```python
from build123d import *

# Parameters (mm, degrees)
SKETCH_1_W          = 200
SKETCH_1_H          = 200
EXTRUDE_1_DEPTH     = 25
SKETCH_2_W          = 150
SKETCH_2_H          = 150
EXTRUDE_2_DEPTH     = 154
SKETCH_3_R          = 60
EXTRUDE_3_DEPTH     = 154
FILLET_1_R          = 10
SKETCH_4_R          = 50
EXTRUDE_4_DEPTH     = 100
SKETCH_5_R          = 50
SKETCH_5_R_2        = 45
EXTRUDE_5_DEPTH     = 100
SKETCH_6_R          = 48
CUT_EXTRUDE_1_DEPTH = 100


with BuildPart() as part:
    # 草图1 → 凸台-拉伸1 (new body)
    with BuildSketch(Plane.XY):
        Rectangle(SKETCH_1_W, SKETCH_1_H)
    extrude(amount=EXTRUDE_1_DEPTH)

    # 草图2 → 凸台-拉伸2 (add)
    with BuildSketch(Plane.XY.offset(25)):
        Rectangle(SKETCH_2_W, SKETCH_2_H)
    extrude(amount=EXTRUDE_2_DEPTH)

    # 草图3 → 凸台-拉伸3 (add)
    with BuildSketch(Plane(origin=(-75, 0, 0), x_dir=(0, 0, -1), z_dir=(1, 0, 0))):
        with Locations((-105, -5)):
            Circle(SKETCH_3_R)
    extrude(amount=-EXTRUDE_3_DEPTH)

    # 圆角1
    fillet_1_edges = [part.edges().sort_by_distance(p)[0] for p in [
        (-229, -5, 165),
    ]]
    fillet(fillet_1_edges, radius=FILLET_1_R)

    # 草图4 → 凸台-拉伸4 (add)
    with BuildSketch(Plane.XY.offset(179)):
        Circle(SKETCH_4_R)
    extrude(amount=EXTRUDE_4_DEPTH)

    # 草图5 → 凸台-拉伸5 (add)
    with BuildSketch(Plane(origin=(0, 75, 0), x_dir=(1, 0, 0), z_dir=(0, 1, 0))):
        with Locations(Location((0, -85, 0), (0, 0, 90))):
            Circle(SKETCH_5_R)
        with Locations(Location((0, -85, 0), (0, 0, 270))):
            Circle(SKETCH_5_R_2, mode=Mode.SUBTRACT)
    extrude(amount=EXTRUDE_5_DEPTH)

    # 草图6 → 切除-拉伸1 (cut)
    with BuildSketch(Plane.XY.offset(279)):
        Circle(SKETCH_6_R)
    extrude(amount=-CUT_EXTRUDE_1_DEPTH, mode=Mode.SUBTRACT)


solid = part.part
```
Could you check a few things on this model? Use its own coordinates, in mm. A direction names the side the tool comes from. Round coordinates to 2 decimals unless told otherwise and drop trailing zeros. Order: outer loops, then holes, each group sorted by start corner. A loop starts at its lowest first (then second) coordinate and runs counter-clockwise, first axis right, second up. Notation, with made-up numbers: (19.5, -26.5) -> (38.5, -26.5) arc R7 ccw to (38.5, -20.5) -> close; hole circle Ø1 at (8, 20). An arc over 180 degrees is marked (long way). One line per question, with ' | ' between items.
Q1. We'd pull the mould along X, two halves only. Please class faces 1 (the face through (-47.954, 2.11, 229.7)), 2 (the face through (1.979, 124.3, 40.044)), 3 (the face through (-1, 1, 0)), 4 (the face through (47.69, 15.02, 228.3)): released by +X, released by -X, zero draft, split by the parting line, or undercut.
Computed values:
face 1: undercut | face 2: undercut | face 3: zero draft | face 4: split by the parting line
Q2. If we section it at C-C on z = 219: Write out the boundary of the cut face in (x, y), plus the area to 3 significant figures.
Computed values:
outline: circle Ø100 at (0, 0); hole circle Ø96 at (0, 0) | area: 616 mm²
Q3. Which directions (+Z, -Z, +X, -X, +Y, -Y) give clear straight access to the entire face, cutting with the end or side of a thin tool? Please do faces 5 (the face through (-90, 1, 25)), 6 (the face through (-1, 51, 179)), 7 (the face through (-145.99, -2.36, 164.94)).
Computed values:
face 5: none | face 6: +Z | face 7: -X
Q4. If we section it at D-D on y = 113.5: Write out the boundary of the cut face in (x, z).
Computed values:
outline: circle Ø100 at (0, 85); hole circle Ø90 at (0, 85)
Q5. If we section it at A-A on y = 84: Write out the boundary of the cut face in (x, z), plus the area to 3 significant figures.
Computed values:
outline: (-100, 0) -> (100, 0) -> (100, 25) -> (-100, 25) -> close; circle Ø100 at (0, 85); hole circle Ø90 at (0, 85) | area: 6,490 mm²
Q6. I'm going to push flat-ended pins straight in: pin 1 (7.5 mm diameter, centred on x = -22, z = 11, fed in from +Y); pin 2 (3 mm diameter, centred on y = 117, z = 72.5, fed in from -X) (3 decimals); pin 3 (12.5 mm diameter, centred on y = 20.5, z = 9.5, fed in from -X). Where does each tip first touch, or does it pass through?
Computed values:
pin 1: y = 100 | pin 2: x = -48.775 | pin 3: x = -100
Q7. If we section it at B-B on x = 0: Write out the boundary of the cut face in (y, z).
Computed values:
outline: (-100, 0) -> (100, 0) -> (100, 25) -> (75, 25) -> (75, 35) -> (175, 35) -> (175, 40) -> (75, 40) -> (75, 130) -> (175, 130) -> (175, 135) -> (75, 135) -> (75, 179) -> (50, 179) -> (50, 279) -> (48, 279) -> (48, 179) -> (-48, 179) -> (-48, 279) -> (-50, 279) -> (-50, 179) -> (-75, 179) -> (-75, 25) -> (-100, 25) -> close
Q8. If I drill on line 1 (X direction, y = 133.5, z = 85); line 2 (Y direction, x = 2, z = 183); line 3 (Z direction, x = -53.5, y = -79.5), over which ranges is the centre line in solid material (lowest first)? Write a range as from..to.
Computed values:
line 1: -50..-45, 45..50 | line 2: -49.96..-47.96, 47.96..49.96 | line 3: 0..25
